Build history of the part. All positions in model axes, mm. A direction names the side the tool comes from. Round coordinates to 2 decimals unless told otherwise and drop trailing zeros. Loops run counter-clockwise (first coordinate to the right, second up) from the corner with the lowest first, then second, coordinate; pieces in that order, holes last. Notation, with made-up numbers: (-38, 4.5) - (-6, 4.5) arc R14 cw to (-6, 27.5) - close; hole circle Ø9 at (-2.75, 59.5). An arc over 180 degrees is marked (long way). Use a Markdown table: item, result.
from build123d import *

# Parameters (mm, degrees)
SKETCH1_W                      = 150
SKETCH1_H                      = 160
BOSS_EXTRUDE1_DEPTH            = 37.5
SHELL1_T                       = -1.5
F_5_5_5_5_DIAMETER_HOLE2_D     = 5.5
SKETCH6_R                      = 15
CUT_EXTRUDE2_DEPTH             = 181.641218995
SKETCH8_R                      = 2
BOSS_EXTRUDE2_DEPTH            = 3
M5_TAPPED_HOLE1_D              = 4.2
M5_TAPPED_HOLE1_DEPTH          = 14
M5_TAPPED_HOLE1_TIP            = 1.2618073
F_5_5_5_5_DIAMETER_HOLE1_D     = 5.5
F_5_5_5_5_DIAMETER_HOLE1_DEPTH = 15
F_5_5_5_5_DIAMETER_HOLE1_TIP   = 1.652366702


with BuildPart() as part:
    # Sketch1 → Boss-Extrude1 (new, symmetric)
    with BuildSketch(Plane.XY):
        Rectangle(SKETCH1_W, SKETCH1_H)
    extrude(amount=BOSS_EXTRUDE1_DEPTH, both=True)

    # Shell1
    shell1_openings = [part.faces().sort_by_distance(p)[0] for p in [
        (0, 0, 37.5),
    ]]
    offset(amount=SHELL1_T, openings=shell1_openings, kind=Kind.INTERSECTION)

    # Ø5.5 (5.5) Diameter Hole2 (through all)
    with Locations(Plane.XY.offset(-36)):
        with Locations((-30, 42), (-5, -42)):
            Hole(F_5_5_5_5_DIAMETER_HOLE2_D / 2)

    # Sketch6 → Cut-Extrude2 (cut, through all)
    with BuildSketch(Plane(origin=(0, 80, 0), x_dir=(1, 0, 0), z_dir=(0, 1, 0))):
        with Locations(Location((-30, 7.5, 0), (0, 0, 270))):
            Circle(SKETCH6_R)
        with Locations(Location((30, 7.5, 0), (0, 0, 270))):
            Circle(SKETCH6_R)
    extrude(amount=-CUT_EXTRUDE2_DEPTH, mode=Mode.SUBTRACT)

    # Sketch8 → Boss-Extrude2 (add)
    with BuildSketch(Plane(origin=(0, 80, 0), x_dir=(1, 0, 0), z_dir=(0, 1, 0))):
        with Locations(Location((-35, -31.5, 0), (0, 0, 90))):
            Circle(SKETCH8_R)
        with Locations(Location((35, -31.5, 0), (0, 0, 90))):
            Circle(SKETCH8_R)
    extrude(amount=BOSS_EXTRUDE2_DEPTH)

    # M5 Tapped Hole1
    with Locations(Plane.XZ.offset(80)):
        with Locations((0, 31.5)):
            Hole(M5_TAPPED_HOLE1_D / 2, depth=M5_TAPPED_HOLE1_DEPTH)
            with Locations((0, 0, -(M5_TAPPED_HOLE1_DEPTH + M5_TAPPED_HOLE1_TIP / 2))):  # 118° drill point
                Cone(0, M5_TAPPED_HOLE1_D / 2, M5_TAPPED_HOLE1_TIP, mode=Mode.SUBTRACT)

    # Ø5.5 (5.5) Diameter Hole1
    with Locations(Plane.XY.offset(-36)):
        with Locations((0, 65), (-35, 65)):
            Hole(F_5_5_5_5_DIAMETER_HOLE1_D / 2, depth=F_5_5_5_5_DIAMETER_HOLE1_DEPTH)
            with Locations((0, 0, -(F_5_5_5_5_DIAMETER_HOLE1_DEPTH + F_5_5_5_5_DIAMETER_HOLE1_TIP / 2))):  # 118° drill point
                Cone(0, F_5_5_5_5_DIAMETER_HOLE1_D / 2, F_5_5_5_5_DIAMETER_HOLE1_TIP, mode=Mode.SUBTRACT)


solid = part.part
Q1. Cut at C-C, the plane z = -5.5. List the corners of the cut face in (x, y).
Results found:
| item | result |
|---|---|
| outline | (-75, -80) - (-44.87, -80) - (-44.87, -78.5) - (-73.5, -78.5) - (-73.5, 78.5) - (-44.87, 78.5) - (-44.87, 80) - (-75, 80) - close; (-15.13, -80) - (15.13, -80) - (15.13, -78.5) - (-15.13, -78.5) - close; (-15.13, 78.5) - (15.13, 78.5) - (15.13, 80) - (-15.13, 80) - close; (44.87, -80) - (75, -80) - (75, 80) - (44.87, 80) - (44.87, 78.5) - (73.5, 78.5) - (73.5, -78.5) - (44.87, -78.5) - close |
Q2. Pull direction X, two halves, no side cores. Call faces 1 (the face through (-27.973, 43.859, -36.761)), 2 (the face through (-1, 1, -37.5)), 3 (the face through (-75, -1, 1)), 4 (the face through (73.5, -1, 1)): pulls with the +X half, pulls with the -X half, needs draft (parallel to the pull), parting line crosses it, or undercut.
Results found:
| item | result |
|---|---|
| face 1 | undercut |
| face 2 | needs draft |
| face 3 | pulls with the -X half |
| face 4 | undercut |
Q3. Cut at D-D, the plane y = 65. List the corners of the cut face in (x, z).
Results found:
| item | result |
|---|---|
| outline | (-75, -37.5) - (-37.75, -37.5) - (-37.75, -36) - (-73.5, -36) - (-73.5, 37.5) - (-75, 37.5) - close; (-32.25, -37.5) - (-2.75, -37.5) - (-2.75, -36) - (-32.25, -36) - close; (2.75, -37.5) - (75, -37.5) - (75, 37.5) - (73.5, 37.5) - (73.5, -36) - (2.75, -36) - close |
Q4. Drop flat-ended pins along their axis: pin 1 (6.5 mm diameter, centred on x = -30, y = 42, fed in from -Z); pin 2 (7 mm diameter, centred on x = -5, y = -42, fed in from +Z); pin 3 (18 mm diameter, centred on x = 30, z = -7.5, fed in from -Y). Give the stop position or say it passes through.
Results found:
| item | result |
|---|---|
| pin 1 | stops at z = -37.5 |
| pin 2 | stops at z = -36 |
| pin 3 | passes through |
Q5. Cut at B-B, the plane x = -5. List the corners of the cut face in (y, z), plus the area to 3 significant figures.
Results found:
| item | result |
|---|---|
| outline | (-80, -37.5) - (-44.75, -37.5) - (-44.75, -36) - (-78.5, -36) - (-78.5, 37.5) - (-80, 37.5) - close; (-39.25, -37.5) - (80, -37.5) - (80, 37.5) - (78.5, 37.5) - (78.5, -36) - (-39.25, -36) - close |
| area | 452 mm2 |
Q6. Which spindle directions (+Z, -Z, +X, -X, +Y, -Y) get a long thin tool onto all of the face, cutting with end or side? Do faces 5 (the face through (36.774, 81.479, 30.577)), 6 (the face through (0.46, -79.24, 29.45)), 7 (the face through (-1, 78.5, 1)). Say none if no direction does.
Results found:
| item | result |
|---|---|
| face 5 | +Y |
| face 6 | -Y |
| face 7 | +Z |
Q7. Probe line 1 (X direction, y = 79, z = -7); line 2 (X direction, y = -15, z = 23.5); line 3 (Y direction, x = 23, z = 22.5). List the from-to ranges inside material, lowest first.
Results found:
| item | result |
|---|---|
| line 1 | x = -75 to -44.99, -15.01 to 15.01, 44.99 to 75 |
| line 2 | x = -75 to -73.5, 73.5 to 75 |
| line 3 | y = -80 to -78.5, 78.5 to 80 |
Q8. Cut at A-A, the plane y = -42. List the corners of the cut face in (x, z).
Results found:
| item | result |
|---|---|
| outline | (-75, -37.5) - (-7.75, -37.5) - (-7.75, -36) - (-73.5, -36) - (-73.5, 37.5) - (-75, 37.5) - close; (-2.25, -37.5) - (75, -37.5) - (75, 37.5) - (73.5, 37.5) - (73.5, -36) - (-2.25, -36) - close |
